from build123d import *

# Parameters (mm, degrees)
BASE_BLOCK_DEPTH   = 20
HUB_BOSS_DEPTH     = 20
LEG_PROFILE_W      = 60
LEG_PROFILE_H      = 20
LEG_DEPTH          = 20
TOP_ARM_DEPTH      = 20
HUB_BORE_SKETCH_R  = 10
HUB_BORE_CUT_DEPTH = 20
LEG_SLOT_SKETCH_R  = 10
LEG_SLOT_CUT_DEPTH = 20


with BuildPart() as part:
    # Base Block Profile → Base Block (new body)
    with BuildSketch(Plane.XY):
        with BuildLine():
            Line((0, 0), (-85, 0))
            ThreePointArc((-85, 0), (-95.606601718, 4.393398282), (-100, 15))
            Line((-100, 15), (-100, 60))
            Line((-100, 60), (0, 60))
            Line((0, 60), (0, 0))
        make_face()
    extrude(amount=BASE_BLOCK_DEPTH)

    # Hub Boss Profile → Hub Boss (add)
    with BuildSketch(Plane(origin=(0, 0, 0), x_dir=(0, 0, -1), z_dir=(1, 0, 0))):
        with BuildLine():
            Line((-20, 0), (-20, 40))
            Line((-20, 40), (-40, 40))
            Line((-40, 40), (-40, 0))
            Line((-40, 0), (-35, 0))
            Line((-35, 0), (-35, 25))
            ThreePointArc((-35, 25), (-29, 31), (-23, 25))
            Line((-23, 25), (-23, 0))
            Line((-23, 0), (-20, 0))
        make_face()
    extrude(amount=-HUB_BOSS_DEPTH)

    # Leg Profile → Leg (add)
    with BuildSketch(Plane(origin=(0, 60, 0), x_dir=(1, 0, 0), z_dir=(0, 1, 0))):
        with Locations((-70, -30)):
            Rectangle(LEG_PROFILE_W, LEG_PROFILE_H)
    extrude(amount=-LEG_DEPTH)

    # Top Arm Profile → Top Arm (add)
    with BuildSketch(Plane(origin=(0, 60, 0), x_dir=(1, 0, 0), z_dir=(0, 1, 0))):
        with BuildLine():
            Line((-40, -20), (0, -20))
            Line((0, -20), (0, -65))
            ThreePointArc((0, -65), (-20, -85), (-40, -65))
            Line((-40, -65), (-40, -20))
        make_face()
    extrude(amount=-TOP_ARM_DEPTH)

    # Hub Bore Sketch → Hub Bore Cut (cut)
    with BuildSketch(Plane.XZ.offset(-40)):
        with Locations(Location((-20, 65, 0), (0, 0, 270))):
            Circle(HUB_BORE_SKETCH_R)
    extrude(amount=-HUB_BORE_CUT_DEPTH, mode=Mode.SUBTRACT)

    # Leg Slot Sketch → Leg Slot Cut (cut)
    with BuildSketch(Plane.XY.offset(20)):
        with Locations((-75, 20)):
            Circle(LEG_SLOT_SKETCH_R)
    extrude(amount=-LEG_SLOT_CUT_DEPTH, mode=Mode.SUBTRACT)


solid = part.part
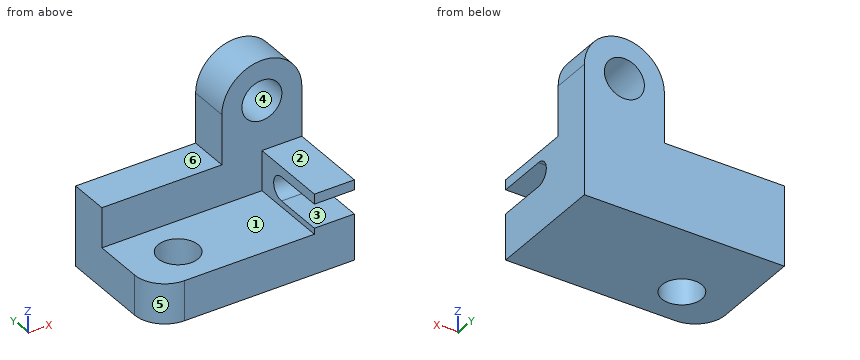
Read the model definition and answer for the solid it produces. Units are mm, in the model's axes. Face numbers are marked on the shaded views. A direction names the side the tool comes from. Round coordinates to 2 decimals unless told otherwise and drop trailing zeros. Loops run counter-clockwise (first coordinate to the right, second up) from the corner with the lowest first, then second, coordinate; pieces in that order, holes last.
Q1. Consider probe 1 along X at (y, z) = (55.5, 65); probe 2 along Y at (x, z) = (-94, 23.5); probe 3 along Y at (x, z) = (-75, 12). Determine where each line is inside the solid, lowest interval first.
Q2. Section D-D on y = 47.5 is taken. Write down the section's boundary in (x, z).
Q3. Each of these flat-tipped pins is pushed along its axis until it touches: pin 1 (2 mm diameter, centred on y = 7.5, z = 34.5, fed in from +X); pin 2 (10 mm diameter, centred on y = 14, z = 33, fed in from -X); pin 3 (10 mm diameter, centred on x = -11, y = 13, fed in from +Z); pin 4 (6 mm diameter, centred on x = -21, z = 59, fed in from +Y). Where does it stop, or does it pass through?
Q4. Section A-A on y = 20 is taken. Write down the section's boundary in (x, z), and give its area (3 significant figures).
Q5. Section B-B on x = -75 is taken. Write down the section's boundary in (y, z).
Q6. Which of the six approach directions +Z, -Z, +X, -X, +Y, -Y give full straight-line access (tool end or side, diameter ignored) to the marked faces 1, 2 and 3?
Q7. Section C-C on z = 60 is taken. Write down the section's boundary in (x, y).
Q8. Determine the mould class of the marked faces 4, 5 and 6 for opening direction X: released by +X, released by -X, zero draft, split by the parting line, or undercut.
Output:
1. probe 1: x = -40 to -30, -10 to 0
1. probe 2: y = 40 to 60
1. probe 3: y = 0 to 10, 30 to 60
2. outline: (-100, 0) - (0, 0) - (0, 65) arc R20 ccw to (-40, 65) - (-40, 40) - (-100, 40) - close; hole circle Ø20 at (-20, 65)
3. pin 1: stops at x = 0
3. pin 2: stops at x = -20
3. pin 3: stops at z = 40
3. pin 4: passes through
4. outline: (-100, 0) - (-85, 0) - (-85, 20) - (-100, 20) - close; (-65, 0) - (0, 0) - (0, 23) - (-20, 23) - (-20, 20) - (-65, 20) - close; (-20, 35) - (0, 35) - (0, 40) - (-20, 40) - close
4. area: 1,760 mm2
5. outline: (0, 0) - (10, 0) - (10, 20) - (0, 20) - close; (30, 0) - (60, 0) - (60, 40) - (40, 40) - (40, 20) - (30, 20) - close
6. face 1: +Z, -X, -Y
6. face 2: +Z, +X, -X, -Y
6. face 3: +X, -X, -Y
7. outline: (-40, 40) - (-28.66, 40) - (-28.66, 60) - (-40, 60) - close; (-11.34, 40) - (0, 40) - (0, 60) - (-11.34, 60) - close
8. face 4: undercut
8. face 5: released by -X
8. face 6: zero draft
